Geometry check sheet. Reference: the model listing, model coordinates, mm. Face numbers are marked on the shaded views. Give positions to 0.01 mm unless a question says otherwise; leave off trailing zeros. Loops run counter-clockwise (first coordinate to the right, second up) from the corner with the lowest first, then second, coordinate; pieces in that order, holes last. Notation, with made-up numbers: (49, 37.25) - (67, 37.25) arc R18 ccw to (67, 47.25) - close; hole circle Ø3 at (34, 63). An arc over 180 degrees is marked (long way). Use a Markdown table: item, result. Add a question column.
1. Material ranges on L1, parallel to Z at x = 685, y = 17.25; L2, parallel to X at y = 14.25, z = -671; L3, parallel to Z at x = 531, y = 2.75, recorded low to high.
2. Draft check along X on the marked faces 1 and 2. Enter one of: pulls with the +X half, pulls with the -X half, needs draft (parallel to the pull), parting line crosses it, or undercut.
3. Cross-section at B-B on y = 4. Count the separate pieces of the cut face and the enclosed holes in it, and give its area (3 significant figures).
4. Cross-section at A-A on x = 37. Enter the section's corners in (y, z).
5. Depth check by flat-ended pin: P1, Ø6, axis at y = 9.5, z = -421, coming from the -X side; P2, Ø8, axis at y = 10.5, z = -515.5, coming from the +X side; P3, Ø8, axis at y = 21.5, z = 313.5, coming from the +X side. Enter the tip coordinate at first touch or a pass-through.
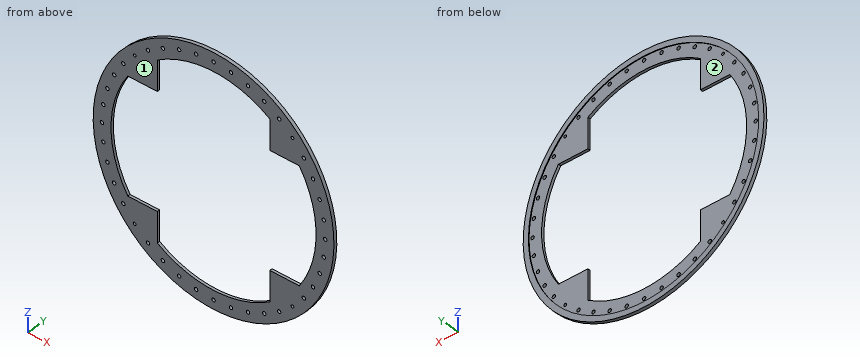
from build123d import *

# Parameters (mm, degrees)
SKETCH_1_R               = 910
EXTRUDE_1_DEPTH          = 25
SKETCH_2_R               = 870
CUT_EXTRUDE_1_DEPTH      = 5
HOLE_WIZARD_26_1_D       = 26
PATTERN_CIRCULAR_1_COUNT = 40
HOLE_WIZARD_M24_1_D      = 21


with BuildPart() as part:
    # 草图1 → 凸台-拉伸1 (new body)
    with BuildSketch(Plane(origin=(0, 0, 0), x_dir=(1, 0, 0), z_dir=(0, 1, 0))):
        with Locations(Location((0, 0, 0), (0, 0, 270))):
            Circle(SKETCH_1_R)
        with BuildLine():
            Line((-648.074069841, 425), (-425, 425))
            Line((-425, 425), (-425, 648.074069841))
            ThreePointArc((-425, 648.074069841), (0, 775), (425, 648.074069841))
            Line((425, 648.074069841), (425, 425))
            Line((425, 425), (648.074069841, 425))
            ThreePointArc((648.074069841, 425), (775, 0), (648.074069841, -425))
            Line((648.074069841, -425), (425, -425))
            Line((425, -425), (425, -648.074069841))
            ThreePointArc((425, -648.074069841), (0, -775), (-425, -648.074069841))
            Line((-425, -648.074069841), (-425, -425))
            Line((-425, -425), (-648.074069841, -425))
            ThreePointArc((-648.074069841, -425), (-775, 0), (-648.074069841, 425))
        make_face(mode=Mode.SUBTRACT)
    extrude(amount=EXTRUDE_1_DEPTH)

    # 草图2 → 切除-拉伸1 (cut)
    with BuildSketch(Plane(origin=(0, 25, 0), x_dir=(1, 0, 0), z_dir=(0, 1, 0))):
        with Locations(Location((0, 0, 0), (0, 0, 270))):
            Circle(SKETCH_2_R)
    extrude(amount=-CUT_EXTRUDE_1_DEPTH, mode=Mode.SUBTRACT)

    # Ø26 直径孔1 (through all)
    with Locations(Plane(origin=(0, 20, 0), x_dir=(1, 0, 0), z_dir=(0, 1, 0))):
        with Locations((0, 843.5)):
            hole_wizard_26_1 = Hole(HOLE_WIZARD_26_1_D / 2)

    # 阵列(圆周)1: Ø26 直径孔1 ×40 about axis, 4 skipped
    pattern_circular_1_axis = Axis((0, 0, 0), (0, 1, 0))
    add([hole_wizard_26_1.rotate(pattern_circular_1_axis, i * 360 / PATTERN_CIRCULAR_1_COUNT) for i in range(1, PATTERN_CIRCULAR_1_COUNT) if i not in (5, 15, 25, 35)], mode=Mode.SUBTRACT)

    # M24 螺纹孔1 (through all)
    with Locations(Plane(origin=(0, 20, 0), x_dir=(1, 0, 0), z_dir=(0, 1, 0))):
        with Locations((-596.444569931, 596.444569931), (596.444569931, 596.444569931), (596.444569931, -596.444569931), (-596.444569931, -596.444569931)):
            Hole(HOLE_WIZARD_M24_1_D / 2)


solid = part.part
Values found:
| question | item | result |
|---|---|---|
| 1 | L1 | z = -599.06 to -508.54, -483.06 to -362.49, 362.49 to 483.06, 508.54 to 599.06 |
| 1 | L2 | x = -614.7 to -502.03, -489.56 to -387.79, 387.79 to 489.56, 502.03 to 614.7 |
| 1 | L3 | z = -739.01 to -425, 425 to 739.01 |
| 2 | face 1 | needs draft |
| 2 | face 2 | undercut |
| 3 | separate pieces | 1 |
| 3 | enclosed holes | 41 |
| 3 | area | 807,000 mm2 |
| 4 | outline | (0, -909.25) - (25, -909.25) - (25, -869.21) - (20, -869.21) - (20, -774.12) - (0, -774.12) - close; (0, 774.12) - (20, 774.12) - (20, 869.21) - (25, 869.21) - (25, 909.25) - (0, 909.25) - close |
| 5 | P1 | stops at x = -808.32 |
| 5 | P2 | stops at x = 752.64 |
| 5 | P3 | stops at x = 855.75 |
